Source: CAD feature listing. Evaluate the final solid. Frame: model axes, mm. A direction names the side the tool comes from. Coordinates: 2 decimals unless noted, no trailing zeros. Order: outer loops, then holes, each group sorted by start corner. A loop starts at its lowest first (then second) coordinate and runs counter-clockwise, first axis right, second up.
Item 1: Section C-C on x = -5.5. Return the cut outline in (y, z), then the cut area to 3 significant figures.
Item 2: Section B-B on z = 1.5. Return the cut outline in (x, y).
Item 3: Section A-A on y = 265. Return the cut outline in (x, z), then the cut area to 3 significant figures.
Item 4: Ray query, line 1 (Z direction, x = -12, y = 557); line 2 (Z direction, x = -23, y = 456). Return the intervals inside material, ascending.
Item 5: Reachability of faces 4 (the flat face through (-30, 766, 0)), 5 (the flat face through (26, 727, 0)) from +Z, -Z, +X, -X, +Y, -Y: full face, straight path, thin tool, end or side. Return the list, or none.
Item 6: Mould query, pull axis X, two halves, no side actions, for faces 1 (the flat face through (0, 729, -26)), 2 (the flat face through (0, 729, 30)), 3 (the flat face through (-0.4, 1452, -27.1)). Classes: released by +X, released by -X, zero draft, split by the parting line, or undercut.
from build123d import *

# Parameters (mm, degrees)
GB_T_6728_2002_SQUARE_HOLLOW_SECTION_60_DEPTH = 1468
CUT_EXTRUDE1_DEPTH                            = 1470.531898259
CUT_EXTRUDE1_DEPTH_BACK                       = 1470.531898259


with BuildPart() as part:
    # Sketch1 → GB/T 6728-2002 square hollow section 60×60×4(1) (new body)
    with BuildSketch(Plane(origin=(0, 0, 0), x_dir=(-1, 0, 0), z_dir=(0, 1, 0))):
        with BuildLine():
            Line((-22, -30), (22, -30))
            ThreePointArc((22, -30), (27.656854249, -27.656854249), (30, -22))
            Line((30, -22), (30, 22))
            ThreePointArc((30, 22), (27.656854249, 27.656854249), (22, 30))
            Line((22, 30), (-22, 30))
            ThreePointArc((-22, 30), (-27.656854249, 27.656854249), (-30, 22))
            Line((-30, 22), (-30, -22))
            ThreePointArc((-30, -22), (-27.656854249, -27.656854249), (-22, -30))
        make_face()
        with BuildLine():
            Line((-22, -26), (22, -26))
            ThreePointArc((22, -26), (24.828427125, -24.828427125), (26, -22))
            Line((26, -22), (26, 22))
            ThreePointArc((26, 22), (24.828427125, 24.828427125), (22, 26))
            Line((22, 26), (-22, 26))
            ThreePointArc((-22, 26), (-24.828427125, 24.828427125), (-26, 22))
            Line((-26, 22), (-26, -22))
            ThreePointArc((-26, -22), (-24.828427125, -24.828427125), (-22, -26))
        make_face(mode=Mode.SUBTRACT)
    extrude(amount=GB_T_6728_2002_SQUARE_HOLLOW_SECTION_60_DEPTH)

    # Sketch2 → Cut-Extrude1 (cut, two sides: drawn at the far end of the back side and taken through both)
    with BuildSketch(Plane.XY.offset(30).offset(-CUT_EXTRUDE1_DEPTH_BACK)):
        Polygon((-30, 0), (-30, 114), (30, 0), align=None)
        Polygon((-30, 1436.421052632), (30, 1468), (-30, 1468), align=None)
    extrude(amount=CUT_EXTRUDE1_DEPTH + CUT_EXTRUDE1_DEPTH_BACK, mode=Mode.SUBTRACT)


solid = part.part
Answer list:
1. outline: (67.45, -30) - (1449.32, -30) - (1449.32, -26) - (67.45, -26) - close; (67.45, 26) - (1449.32, 26) - (1449.32, 30) - (67.45, 30) - close
1. area: 11,100 mm2
2. outline: (-30, 114) - (-26, 106.4) - (-26, 1438.53) - (-30, 1436.42) - close; (26, 7.6) - (30, 0) - (30, 1468) - (26, 1465.89) - close
3. outline: (-30, -22) arc R8 ccw to (-22, -30) - (22, -30) arc R8 ccw to (30, -22) - (30, 22) arc R8 ccw to (22, 30) - (-22, 30) arc R8 ccw to (-30, 22) - close; hole (-26, -22) arc R4 ccw to (-22, -26) - (22, -26) arc R4 ccw to (26, -22) - (26, 22) arc R4 ccw to (22, 26) - (-22, 26) arc R4 ccw to (-26, 22) - close
3. area: 855 mm2
4. line 1: z = -30 to -26, 26 to 30
4. line 2: z = -29.94 to -25.87, 25.87 to 29.94
5. face 4: +Z, -Z, -X, +Y, -Y
5. face 5: +Y, -Y
6. face 1: undercut
6. face 2: zero draft
6. face 3: released by -X
